from build123d import *

# Parameters (mm, degrees)
CHAMFER_2_SIZE           = 1
CUT_EXTRUDE_1_DEPTH      = 49.38129804
CUT_EXTRUDE_1_DEPTH_BACK = 49.38129804
SKETCH_2_W               = 1.5
SKETCH_2_H               = 2
SKETCH_3_R               = 5.5
CUT_EXTRUDE_2_DEPTH      = 10


with BuildPart() as part:
    # 草图1 → 旋转1 (revolve)
    with BuildSketch(Plane.XY, mode=Mode.PRIVATE) as revolve_1_sk:
        Polygon((0, 0), (0, 6.5), (3.5, 6.5), (3.5, 5), (47.5, 5), (47.5, 0), align=None)
    revolve(revolve_1_sk.sketch.rotate(Axis((-19.421134541, 0, 0), (1, 0, 0)), 90), axis=Axis((-19.421134541, 0, 0), (1, 0, 0)))

    # 倒角2
    chamfer_2_edges = [part.edges().sort_by_distance(p)[0] for p in [
        (47.5, 0, -5),
    ]]
    chamfer(chamfer_2_edges, length=CHAMFER_2_SIZE)

    # 草图2 → 切除-拉伸1 (cut, two sides: drawn at the far end of the back side and taken through both)
    with BuildSketch(Plane.XY.offset(-CUT_EXTRUDE_1_DEPTH_BACK)):
        with Locations((0.75, 0)):
            Rectangle(SKETCH_2_W, SKETCH_2_H)
    extrude(amount=CUT_EXTRUDE_1_DEPTH + CUT_EXTRUDE_1_DEPTH_BACK, mode=Mode.SUBTRACT)

    # 草图3 → 切除-拉伸2 (cut)
    with BuildSketch(Plane(origin=(47.5, 0, 0), x_dir=(0, 0, -1), z_dir=(1, 0, 0))):
        Circle(SKETCH_3_R)
    extrude(amount=-CUT_EXTRUDE_2_DEPTH, mode=Mode.SUBTRACT)


solid = part.part
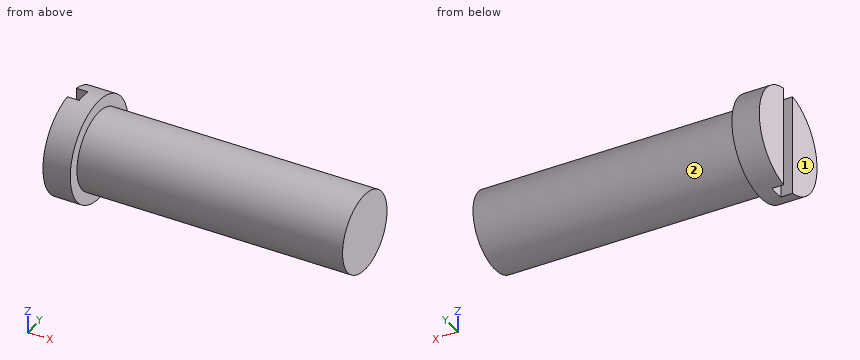
Read the model definition and answer for the solid it produces. Units are mm, in the model's axes. Face numbers are marked on the shaded views. A direction names the side the tool comes from. Give positions to 0.01 mm unless a question says otherwise; leave off trailing zeros. Write each loop counter-clockwise with the first axis right and the second up, starting at its lowest first coordinate (ties: lowest second). Pieces come first, ordered by that corner, then holes. Notation, with made-up numbers: (1, 75.5) - (9, 75.5) arc R26 ccw to (9, 113.5) - close; hole circle Ø8 at (75.25, -31.5). An arc over 180 degrees is marked (long way). Use CSV: the item, a comma, the result in double quotes. Start each with the question number.
(1) Consider line 1 along X through (y, z) = (-4.75, -4); line 2 along Z through (x, y) = (4, -3); line 3 along Z through (x, y) = (13, -2). Determine where each line is inside the solid, lowest interval first.
(2) Find section A-A (z = 0). Give the vertices of the cut face in (x, y).
(3) Find section B-B (y = 0). Give the vertices of the cut face in (x, z), plus the area to 3 significant figures.
(4) Given P1, Ø5, axis at x = 32.5, y = 1, coming from the +Z side; P2, Ø1.5, axis at x = 7, z = -4.5, coming from the +Y side; P3, Ø1.5, axis at x = 24, z = 0, coming from the +Y side, each flat-ended and moving along its own axis, determine where each tip first touches the part or whether it passes through.
(5) For the marked faces 1 and 2, determine the directions among +Z, -Z, +X, -X, +Y, -Y from which every point of the face is accessible in a straight line to the end or side of a thin tool.
(6) Find section D-D (z = 2.75). Give the vertices of the cut face in (x, y), plus the area to 3 significant figures.
(7) Find section C-C (x = 10). Give the vertices of the cut face in (y, z), plus the area to 3 significant figures.
Findings below:
1,line 1,"0 to 3.5"
1,line 2,"-4 to 4"
1,line 3,"-4.58 to 4.58"
2,outline,"(0, -6.5) - (3.5, -6.5) - (3.5, -5) - (37.5, -5) - (37.5, 5) - (3.5, 5) - (3.5, 6.5) - (0, 6.5) - (0, 1) - (1.5, 1) - (1.5, -1) - (0, -1) - close"
3,outline,"(1.5, -6.5) - (3.5, -6.5) - (3.5, -5) - (37.5, -5) - (37.5, 5) - (3.5, 5) - (3.5, 6.5) - (1.5, 6.5) - close"
3,area,"366 mm2"
4,P1,"z = 5"
4,P2,"y = 3.31"
4,P3,"y = 5"
5,face 1,"+Z, -Z, -X, +Y, -Y"
5,face 2,"+X"
6,outline,"(0, -5.89) - (3.5, -5.89) - (3.5, -4.18) - (37.5, -4.18) - (37.5, 4.18) - (3.5, 4.18) - (3.5, 5.89) - (0, 5.89) - (0, 1) - (1.5, 1) - (1.5, -1) - (0, -1) - close"
6,area,"322 mm2"
7,outline,"circle Ø10 at (0, 0)"
7,area,"78.5 mm2"
